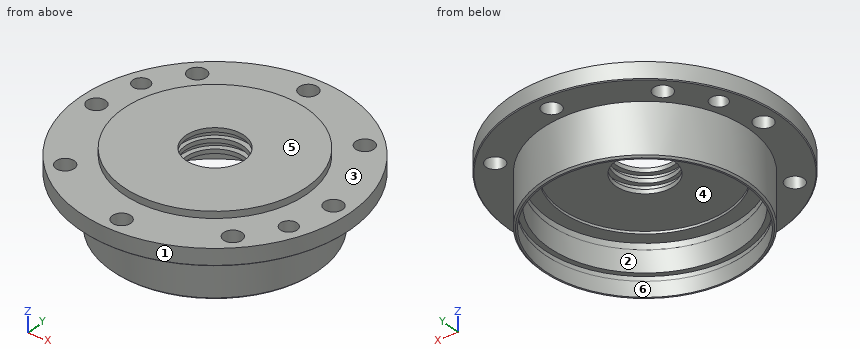
from build123d import *

# Parameters (mm, degrees)
SKETCH1_R                    = 81
BOSS_EXTRUDE1_DEPTH          = 10
SKETCH2_R                    = 55
BOSS_EXTRUDE2_DEPTH          = 4
SKETCH3_R                    = 62
BOSS_EXTRUDE3_DEPTH          = 31
SKETCH4_R                    = 17.5
CUT_EXTRUDE1_DEPTH           = 2.5
SKETCH5_R                    = 20.3
CUT_EXTRUDE2_DEPTH           = 3.5
SKETCH6_R                    = 17.5
CUT_EXTRUDE3_DEPTH           = 2.5
SKETCH7_R                    = 20.3
CUT_EXTRUDE4_DEPTH           = 3.5
SKETCH8_R                    = 17.5
CUT_EXTRUDE5_DEPTH           = 2.5
SKETCH9_R                    = 50
CUT_EXTRUDE6_DEPTH           = 1.5
F_1_0MM_BLIND_DOWEL_HOLE1_D  = 11
CIRPATTERN1_COUNT            = 8
F_10_0MM_BLIND_DOWEL_HOLE1_D = 10
SKETCH18_R                   = 58
CUT_EXTRUDE7_DEPTH           = 4
SKETCH19_R                   = 60
CUT_EXTRUDE8_DEPTH           = 9
SKETCH20_R                   = 60.5
CUT_EXTRUDE9_DEPTH           = 3
CUT_EXTRUDE10_REACH          = 121.21
SKETCH21_R                   = 57.5
CHAMFER1_SIZE                = 1
CHAMFER2_SIZE                = 0.5


with BuildPart() as part:
    # Sketch1 → Boss-Extrude1 (new body)
    with BuildSketch(Plane.XY):
        Circle(SKETCH1_R)
    extrude(amount=BOSS_EXTRUDE1_DEPTH)

    # Sketch2 → Boss-Extrude2 (add)
    with BuildSketch(Plane.XY.offset(10)):
        Circle(SKETCH2_R)
    extrude(amount=BOSS_EXTRUDE2_DEPTH)

    # Sketch3 → Boss-Extrude3 (add)
    with BuildSketch(Plane(origin=(0, 0, 0), x_dir=(-1, 0, 0), z_dir=(0, 0, -1))):
        Circle(SKETCH3_R)
    extrude(amount=BOSS_EXTRUDE3_DEPTH)

    # Sketch4 → Cut-Extrude1 (cut)
    with BuildSketch(Plane.XY.offset(14)):
        Circle(SKETCH4_R)
    extrude(amount=-CUT_EXTRUDE1_DEPTH, mode=Mode.SUBTRACT)

    # Sketch5 → Cut-Extrude2 (cut)
    with BuildSketch(Plane.XY.offset(11.5)):
        Circle(SKETCH5_R)
    extrude(amount=-CUT_EXTRUDE2_DEPTH, mode=Mode.SUBTRACT)

    # Sketch6 → Cut-Extrude3 (cut)
    with BuildSketch(Plane.XY.offset(8)):
        with Locations((-0.303631116, -0.227723337)):
            Circle(SKETCH6_R)
    extrude(amount=-CUT_EXTRUDE3_DEPTH, mode=Mode.SUBTRACT)

    # Sketch7 → Cut-Extrude4 (cut)
    with BuildSketch(Plane.XY.offset(5.5)):
        with Locations((0, 0.379538895)):
            Circle(SKETCH7_R)
    extrude(amount=-CUT_EXTRUDE4_DEPTH, mode=Mode.SUBTRACT)

    # Sketch8 → Cut-Extrude5 (cut)
    with BuildSketch(Plane.XY.offset(2)):
        Circle(SKETCH8_R)
    extrude(amount=-CUT_EXTRUDE5_DEPTH, mode=Mode.SUBTRACT)

    # Sketch9 → Cut-Extrude6 (cut)
    with BuildSketch(Plane.XY.offset(-0.5)):
        Circle(SKETCH9_R)
    extrude(amount=-CUT_EXTRUDE6_DEPTH, mode=Mode.SUBTRACT)

    # Ø1.0mm Blind Dowel Hole1 (through all)
    with Locations(Plane.XY.offset(10)):
        with Locations((0, 71)):
            f_1_0mm_blind_dowel_hole1 = Hole(F_1_0MM_BLIND_DOWEL_HOLE1_D / 2)

    # CirPattern1: Ø1.0mm Blind Dowel Hole1 ×8 about axis
    cirpattern1_axis = Axis((0, 0, 0), (0, 0, 1))
    for i in range(1, CIRPATTERN1_COUNT):
        add(f_1_0mm_blind_dowel_hole1.rotate(cirpattern1_axis, i * 360 / CIRPATTERN1_COUNT), mode=Mode.SUBTRACT)

    # Ø10.0mm Blind Dowel Hole1 (through all)
    with Locations(Plane.XY.offset(10)):
        with Locations((65.595446808, -27.170523698), (-65.595446808, 27.170523698)):
            Hole(F_10_0MM_BLIND_DOWEL_HOLE1_D / 2)

    # Sketch18 → Cut-Extrude7 (cut)
    with BuildSketch(Plane.XY.offset(-2)):
        Circle(SKETCH18_R)
    extrude(amount=-CUT_EXTRUDE7_DEPTH, mode=Mode.SUBTRACT)

    # Sketch19 → Cut-Extrude8 (cut)
    with BuildSketch(Plane(origin=(0, 0, -31), x_dir=(-1, 0, 0), z_dir=(0, 0, -1))):
        Circle(SKETCH19_R)
    extrude(amount=-CUT_EXTRUDE8_DEPTH, mode=Mode.SUBTRACT)

    # Sketch20 → Cut-Extrude9 (cut)
    with BuildSketch(Plane(origin=(0, 0, -22), x_dir=(-1, 0, 0), z_dir=(0, 0, -1))):
        Circle(SKETCH20_R)
    extrude(amount=-CUT_EXTRUDE9_DEPTH, mode=Mode.SUBTRACT)

    # Sketch21 → Cut-Extrude10 (cut, up to next)
    with BuildSketch(Plane(origin=(0, 0, -19), x_dir=(-1, 0, 0), z_dir=(0, 0, -1)), mode=Mode.PRIVATE) as cut_extrude10_sk1:
        Circle(SKETCH21_R)
    cut_extrude10_tool1 = extrude(cut_extrude10_sk1.sketch, amount=-CUT_EXTRUDE10_REACH, mode=Mode.PRIVATE) & part.part
    add(cut_extrude10_tool1.solids().sort_by_distance((0, 0, -19))[0], mode=Mode.SUBTRACT)

    # Chamfer1
    chamfer1_edges = [part.edges().sort_by_distance(p)[0] for p in [
        (62, 0, -31),
    ]]
    chamfer(chamfer1_edges, length=CHAMFER1_SIZE)

    # Chamfer2
    chamfer2_edges = [part.edges().sort_by_distance(p)[0] for p in [
        (-81, 0, 0),
    ]]
    chamfer(chamfer2_edges, length=CHAMFER2_SIZE)


solid = part.part
Geometry: final body of the model. Coordinates: model frame, mm. Face numbers are marked on the shaded views. A direction names the side the tool comes from. Round coordinates to 2 decimals unless told otherwise and drop trailing zeros. Loops run counter-clockwise (first coordinate to the right, second up) from the corner with the lowest first, then second, coordinate; pieces in that order, holes last. Notation, with made-up numbers: M -25,-16.5 L 12,-16.5 A27 cw 12,13.5 Z; hole C -13,78.5 d5. An arc over 180 degrees is marked long. One line per question, with ' | ' between items.
(1) Contact query for flat-ended pins moving along their axis: P1, Ø12, axis at x = -20, z = -5, coming from the -Y side; P2, Ø2, axis at y = 45.5, z = -13, coming from the +X side; P3, Ø6.5, axis at x = 50.2, y = 50.2, coming from the +Z side; P4, Ø11.5, axis at x = 65.6, y = -27.17, coming from the -Z side. Output: stop coordinate, or through.
Check result:
P1: stops at y = -79.06 | P2: stops at x = 43.17 | P3: passes through | P4: stops at z = 0
(2) Cut plane B-B on x = 68.5. Give the number of separate pieces and of enclosed holes in the cut face, plus the area to 3 significant figures.
Check result:
separate pieces: 3 | enclosed holes: 0 | area: 685 mm2
(3) Material intervals for line 1 along Y through (x, z) = (0, 5); line 2 along Y through (x, z) = (0, 9.35); line 3 along Z through (x, y) = (1, -34.5), sorted ascending. Write a range as from..to.
Check result:
line 1: y = -81..-76.5, -65.5..-19.92, 20.68..65.5, 76.5..81 | line 2: y = -81..-76.5, -65.5..-20.3, 20.3..65.5, 76.5..81 | line 3: z = -0.5..14
(4) Access query for the marked faces 5 and 6. Directions: +Z, -Z, +X, -X, +Y, -Y. A direction counts if a zero-diameter tool reaches every point of the face in a straight line with its end or side. Return the directions, or none.
Check result:
face 5: +Z, +X, -X, +Y, -Y | face 6: -Z
(5) Cut plane C-C on z = -27.5. Return the cut outline in (x, y).
Check result:
outline: C 0,0 d124; hole C 0,0 d120
(6) Cut plane A-A on z = -9. Return the cut outline in (x, y), plus the area to 3 significant figures.
Check result:
outline: C 0,0 d124; hole C 0,0 d115 | area: 1,690 mm2
(7) Pull-direction query (Y, two-part tool) for the marked faces 1, 2, 3 and 4; classes: +Y half, -Y half, draft (parallel to the pull), parting line (faces both ways), or undercut.
Check result:
face 1: parting line | face 2: undercut | face 3: draft | face 4: undercut
